```python
from build123d import *

# Parameters (mm, degrees)
SKETCH2_R                  = 10
CUT_EXTRUDE1_DEPTH         = 86.635856976
SKETCH3_W                  = 0.7
SKETCH3_H                  = 1.2
M8_TAPPED_HOLE1_D          = 6.8
F_10_0_10_DIAMETER_HOLE1_D = 10
CHAMFER1_SIZE              = 0.5


with BuildPart() as part:
    # Sketch1 → Revolve1 (revolve)
    with BuildSketch(Plane.XY, mode=Mode.PRIVATE) as revolve1_sk:
        Polygon((0, 0), (42.5, 0), (42.5, 12), (20, 12), (20, 21), (15, 21), (15, 61), (0, 61), align=None)
    revolve(revolve1_sk.sketch.rotate(Axis((0, 0, 0), (0, 1, 0)), 90), axis=Axis((0, 0, 0), (0, 1, 0)))

    # Sketch2 → Cut-Extrude1 (cut, through all)
    with BuildSketch(Plane(origin=(0, 61, 0), x_dir=(1, 0, 0), z_dir=(0, 1, 0))):
        with Locations(Location((0, 0, 0), (0, 0, 270))):
            Circle(SKETCH2_R)
    extrude(amount=-CUT_EXTRUDE1_DEPTH, mode=Mode.SUBTRACT)

    # Sketch3 → Cut-Revolve1 (revolve, cut)
    with BuildSketch(Plane.XY, mode=Mode.PRIVATE) as cut_revolve1_sk:
        with Locations((14.65, 50.6)):
            Rectangle(SKETCH3_W, SKETCH3_H)
    revolve(cut_revolve1_sk.sketch.rotate(Axis((0, 0, 0), (0, -1, 0)), 270), axis=Axis((0, 0, 0), (0, -1, 0)), mode=Mode.SUBTRACT)

    # M8 Tapped Hole1 (through all)
    with Locations(Plane(origin=(0, 12, 0), x_dir=(1, 0, 0), z_dir=(0, 1, 0))):
        with Locations((35, 0), (0, -35), (-35, 0), (0, 35), (0, 0)):
            Hole(M8_TAPPED_HOLE1_D / 2)

    # Ø10.0 (10) Diameter Hole1 (through all)
    with Locations(Plane(origin=(0, 12, 0), x_dir=(1, 0, 0), z_dir=(0, 1, 0))):
        with Locations((-21.213203436, -21.213203436), (21.213203436, 21.213203436)):
            Hole(F_10_0_10_DIAMETER_HOLE1_D / 2)

    # Chamfer1
    chamfer1_edges = [part.edges().sort_by_distance(p)[0] for p in [
        (0, 61, -10),
        (0, 61, 15),
        (0, 12, 42.5),
        (0, 0, 42.5),
    ]]
    chamfer(chamfer1_edges, length=CHAMFER1_SIZE)


solid = part.part
```
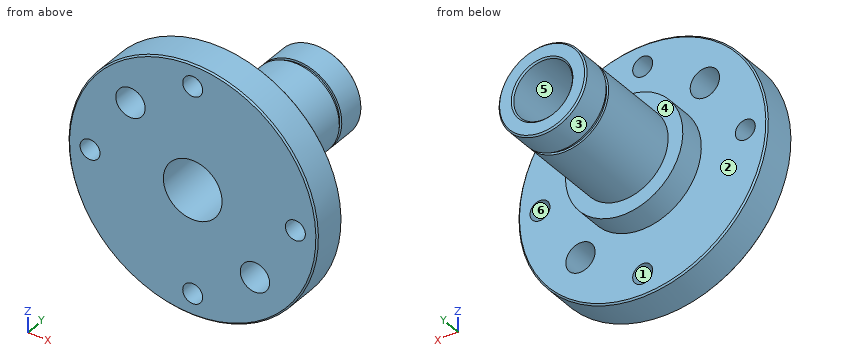
Work out the finished part from the listing and answer in its coordinate system (mm). Face numbers are marked on the shaded views. A direction names the side the tool comes from. Give positions to 0.01 mm unless a question says otherwise; leave off trailing zeros. Loops run counter-clockwise (first coordinate to the right, second up) from the corner with the lowest first, then second, coordinate; pieces in that order, holes last. Notation, with made-up numbers: (54, 37) -> (113, 37) arc R14 cw to (113, 58) -> close; hole circle Ø5 at (9, 54). An arc over 180 degrees is marked (long way). One line per question, with ' | ' between items. Start each with the question number.
1) For the marked faces 1 and 2, determine the directions among +Z, -Z, +X, -X, +Y, -Y from which every point of the face is accessible in a straight line to the end or side of a thin tool.
2) Each of these flat-tipped pins is pushed along its axis until it touches: pin 1 (9 mm diameter, centred on x = 0, z = -35, fed in from +Y); pin 2 (8 mm diameter, centred on x = 21.21, z = -21.21, fed in from +Y); pin 3 (3 mm diameter, centred on y = 12, z = 15, fed in from +X); pin 4 (6 mm diameter, centred on x = -5.5, y = 37, fed in from -Z). Where does it stop, or does it pass through?
3) Section B-B, the plane y = 34.5 is taken. Determine the outline of the cut face in (x, z).
4) Straight lines are drawn through the part: L1, parallel to X at y = 15, z = 0; L2, parallel to Y at x = -30, z = -7.5; L3, parallel to Z at x = 1.5, y = 41.5. For each, find the intervals that lie inside material, in ascending order.
5) Section A-A, the plane y = 4 is taken. Determine the outline of the cut face in (x, z).
6) Determine the mould class of the marked faces 3, 4, 5 and 6 for opening direction Z: +Z half, -Z half, draft (parallel to the pull), parting line (faces both ways), or undercut.
7) Section C-C, the plane x = 0 is taken. State how many separate pieces and enclosed holes the cut face has, then the cut area to 3 significant figures.
Resolved:
1) face 1: +Y, -Y | face 2: +Y
2) pin 1: y = 12 | pin 2: through | pin 3: x = 40.27 | pin 4: z = -14.79
3) outline: circle Ø30 at (0, 0); hole circle Ø20 at (0, 0)
4) L1: -20 to -10, 10 to 20 | L2: 0 to 12 | L3: -14.92 to -9.89, 9.89 to 14.92
5) outline: circle Ø85 at (0, 0); hole circle Ø6.8 at (-35, 0); hole circle Ø10 at (-21.21, 21.21); hole circle Ø20 at (0, 0); hole circle Ø6.8 at (0, -35); hole circle Ø6.8 at (0, 35); hole circle Ø10 at (21.21, -21.21); hole circle Ø6.8 at (35, 0)
6) face 3: parting line | face 4: draft | face 5: undercut | face 6: undercut
7) separate pieces: 4 | enclosed holes: 0 | area: 1,190 mm2
